Here's the drawing with two shaded views (mm, measured from the low corner). I have some questions. Give positions to 0.01 mm unless a question says otherwise; leave off trailing zeros. Write each loop counter-clockwise with the first axis right and the second up, starting at its lowest first coordinate (ties: lowest second). Pieces come first, ordered by that corner, then holes. Notation, with made-up numbers: (28, 33) - (43, 33) arc R31 cw to (43, 70) - close; hole circle Ø8 at (21.5, 44.25). An arc over 180 degrees is marked (long way). Write item = value, one per line.
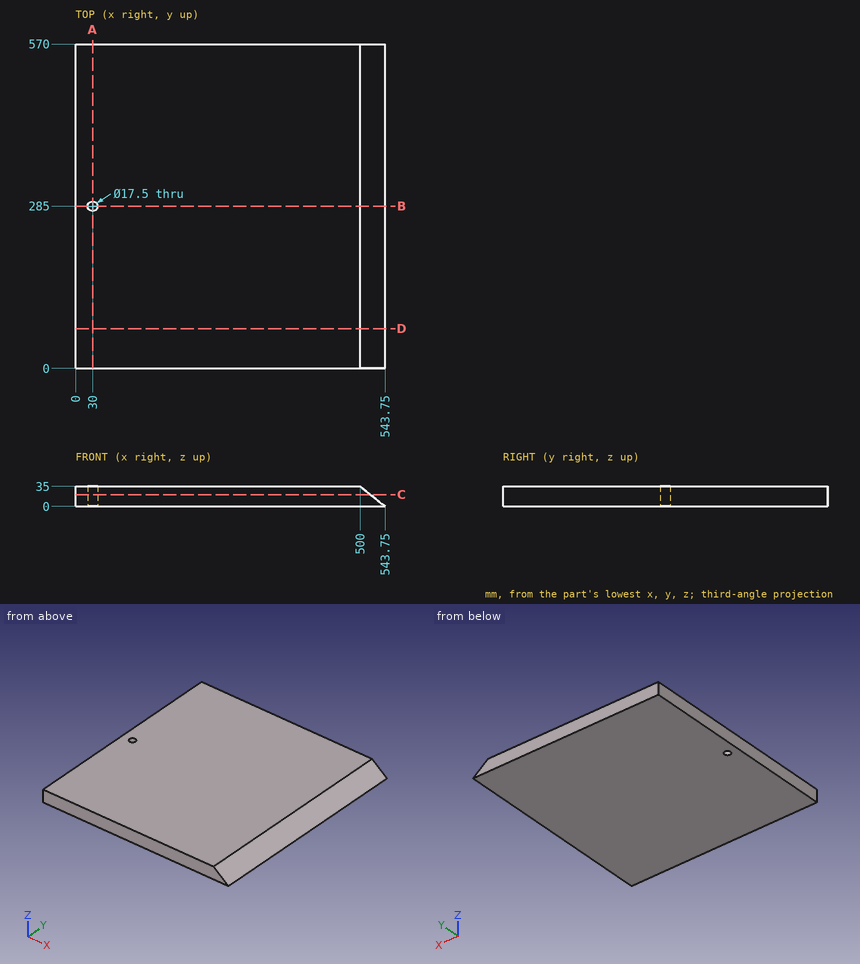
1. If we section it at B-B, the plane y = 285: Please give me the cut outline in (x, z), and give its area (3 significant figures).
Filled sheet:
outline = (0, 0) - (21.25, 0) - (21.25, 35) - (0, 35) - close; (38.75, 0) - (543.75, 0) - (500, 35) - (38.75, 35) - close
area = 17,700 mm2
2. I need wall thicknesses on line 1 (Y direction, x = 30, z = 8.5); line 2 (X direction, y = 40, z = 23); line 3 (X direction, y = 332.5, z = 9). Which ranges of each line are inside material? Lowest first, please.
Filled sheet:
line_1 = 0 to 276.25, 293.75 to 570
line_2 = 0 to 515
line_3 = 0 to 532.5
3. If we section it at C-C, the plane z = 20.5: Please give me the cut outline in (x, y) (3 decimals), and give its area (3 significant figures).
Filled sheet:
outline = (0, 0) - (518.125, 0) - (518.125, 570) - (0, 570) - close; hole circle Ø17.5 at (30, 285)
area = 295,000 mm2
4. For pin 1 (12 mm diameter, centred on y = 498.5, z = 27, fed in from +X), with a flat end and sliding along its axis, tell me the tip position at first contact or that it passes through.
Filled sheet:
pin_1 = 517.5
5. If we section it at A-A, the plane x = 30: Please give me the cut outline in (y, z), and give its area (3 significant figures).
Filled sheet:
outline = (0, 0) - (276.25, 0) - (276.25, 35) - (0, 35) - close; (293.75, 0) - (570, 0) - (570, 35) - (293.75, 35) - close
area = 19,300 mm2
6. If we section it at D-D, the plane y = 70: Please give me the cut outline in (x, z), and give its area (3 significant figures).
Filled sheet:
outline = (0, 0) - (543.75, 0) - (500, 35) - (0, 35) - close
area = 18,300 mm2
